from build123d import *

# Parameters (mm, degrees)
CHAMFER1_SIZE = 0.5


with BuildPart() as part:
    # Sketch1 → Revolve1 (revolve)
    with BuildSketch(Plane(origin=(0, 0, 0), x_dir=(0, 0, -1), z_dir=(1, 0, 0))):
        Polygon((0, 13), (6.25, 13), (6.25, 3), (7.5, 3), (7.5, 0), (0, 0), align=None)
    revolve(axis=Axis((0, 0, 0), (0, 1, 0)))

    # Chamfer1
    chamfer1_edges = [part.edges().sort_by_distance(p)[0] for p in [
        (0, 0, 7.5),
        (0, 3, 7.5),
        (0, 13, 6.25),
    ]]
    chamfer(chamfer1_edges, length=CHAMFER1_SIZE)


solid = part.part
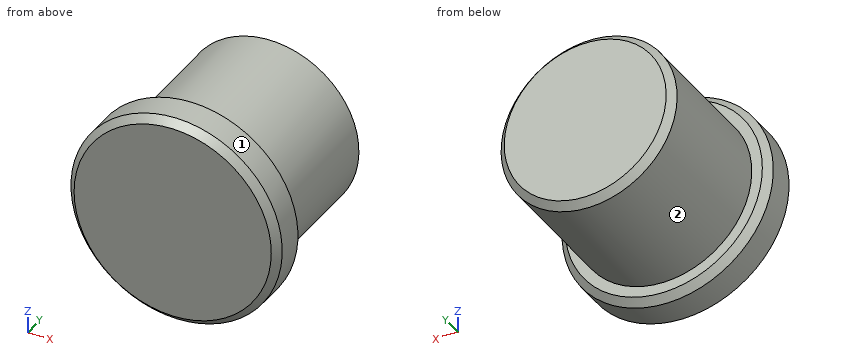
The listing builds one solid part. Answer for the finished solid, in the listing's coordinates (mm). Face numbers are marked on the shaded views. A direction names the side the tool comes from. Round coordinates to 2 decimals unless told otherwise and drop trailing zeros. Order: outer loops, then holes, each group sorted by start corner. A loop starts at its lowest first (then second) coordinate and runs counter-clockwise, first axis right, second up. Notation, with made-up numbers: M 81,17 L 88,17 A22 cw 88,45 Z; hole C 6,86 d4. An arc over 180 degrees is marked long. Answer in a Markdown table with one row per item. Add a question column.
1) The part is cut by section C-C on y = 8. Determine the outline of the cut face in (x, z).
2) The part is cut by section B-B on z = 0. Determine the outline of the cut face in (x, y).
3) Flat-ended cylindrical pins translate along their axes: pin 1 Ø1.5 at (y, z) = (3, -3) entering from -X; pin 2 Ø4 at (x, y) = (4, 10) entering from +Z; pin 3 Ø1 at (x, y) = (-3, 11.5) entering from -Z. Find the tip coordinate at first contact, or state that the pin passes through.
4) Consider line 1 along Y through (x, z) = (6.5, -1.5); line 2 along X through (y, z) = (9.5, -0.25) (3 decimals); line 3 along X through (y, z) = (2.75, 5.5). Determine where each line is inside the solid, lowest interval first. Write a range as from..to.
5) Which of the six approach directions +Z, -Z, +X, -X, +Y, -Y give full straight-line access (tool end or side, diameter ignored) to the marked faces 1 and 2?
6) The part is cut by section A-A on x = 0. Determine the outline of the cut face in (y, z), plus the area to 3 significant figures.
7) The part is cut by section D-D on y = 1. Determine the outline of the cut face in (x, z), plus the area to 3 significant figures.
Findings below:
| question | item | result |
|---|---|---|
| 1 | outline | C 0,0 d12.5 |
| 2 | outline | M -7.5,0.5 L -7,0 L 7,0 L 7.5,0.5 L 7.5,2.5 L 7,3 L 6.25,3 L 6.25,12.5 L 5.75,13 L -5.75,13 L -6.25,12.5 L -6.25,3 L -7,3 L -7.5,2.5 Z |
| 3 | pin 1 | stops at x = -7.09 |
| 3 | pin 2 | stops at z = 5.92 |
| 3 | pin 3 | stops at z = -5.73 |
| 4 | line 1 | y = 0..3 |
| 4 | line 2 | x = -6.245..6.245 |
| 4 | line 3 | x = -4.72..4.72 |
| 5 | face 1 | +Y, -Y |
| 5 | face 2 | +Y |
| 6 | outline | M 0,-7 L 0.5,-7.5 L 2.5,-7.5 L 3,-7 L 3,-6.25 L 12.5,-6.25 L 13,-5.75 L 13,5.75 L 12.5,6.25 L 3,6.25 L 3,7 L 2.5,7.5 L 0.5,7.5 L 0,7 Z |
| 6 | area | 169 mm² |
| 7 | outline | C 0,0 d15 |
| 7 | area | 177 mm² |
